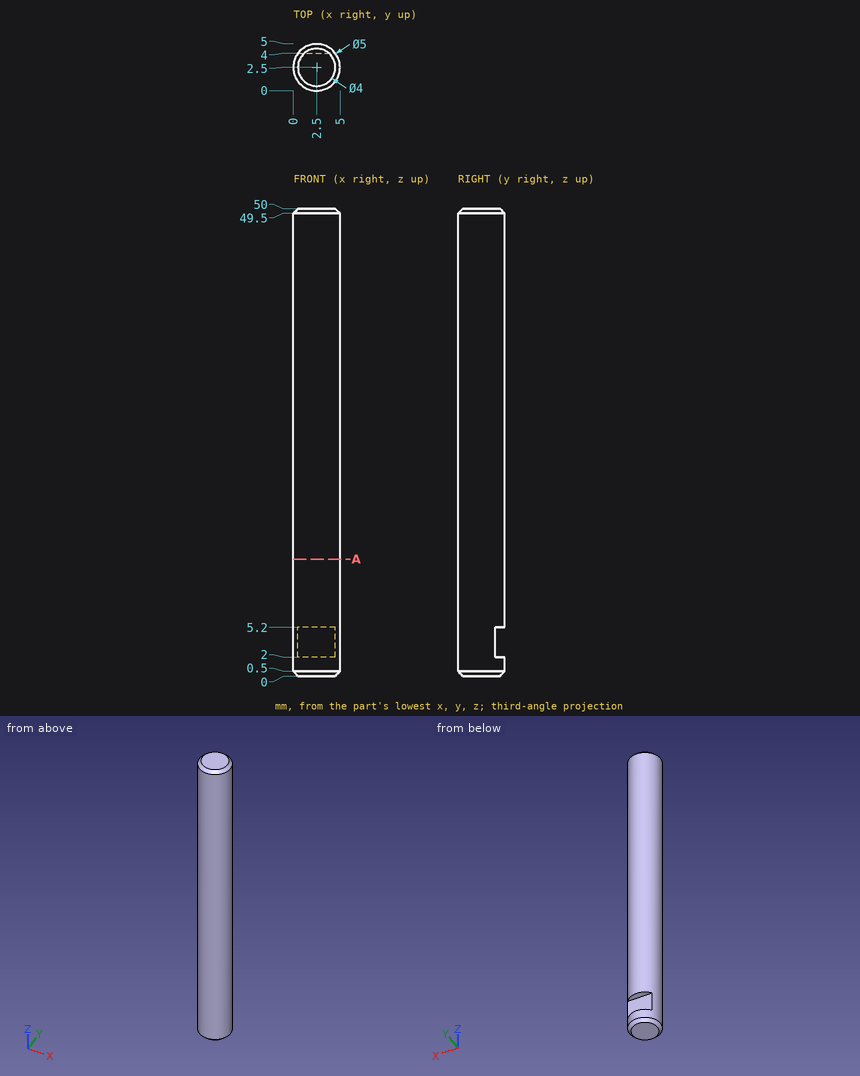
Can you work these out from the drawing? Everything is in mm from the part's minimum corner. Round coordinates to 2 decimals unless told otherwise and drop trailing zeros. Loops run counter-clockwise (first coordinate to the right, second up) from the corner with the lowest first, then second, coordinate; pieces in that order, holes last. Notation, with made-up numbers: (-28, 86.5) -> (0, 86.5) arc R32 cw to (0, 120.5) -> close; hole circle Ø8 at (71, -4). An arc over 180 degrees is marked (long way). Put each result on its own line as item: value.
Q1. I want a section at A-A on z = 12.5. Write out the boundary of the cut face in (x, y), and give its area (3 significant figures).
Checks:
outline: circle Ø5 at (2.5, 2.5)
area: 19.6 mm2
Q2. For pin 1 Ø2.5 at (x, z) = (1.5, 3) entering from +Y; pin 2 Ø1.5 at (y, z) = (1, 39.5) entering from +X; pin 3 Ø0.8 at (x, y) = (3, 4.5) entering from +Z; pin 4 Ø1 at (y, z) = (4, 31) entering from +X, each with a flat end and sliding along its axis, tell me the tip position at first contact or that it passes through.
Checks:
pin 1: y = 4.99
pin 2: x = 4.88
pin 3: z = 50
pin 4: x = 4.79
Q3. Please list where these lines run through material, in increasing order: line 1 (Y direction, x = 2.3, z = 5); line 2 (X direction, y = 2.7, z = 33.5); line 3 (Z direction, x = 0.4, y = 1.75). Write a range as from..to.
Checks:
line 1: 0.01..4
line 2: 0.01..4.99
line 3: 0.23..49.77
